Here's how the part is built. I have some questions about the finished solid (model axes, mm). A direction names the side the tool comes from. Coordinates: 2 decimals unless noted, no trailing zeros. Write each loop counter-clockwise with the first axis right and the second up, starting at its lowest first coordinate (ties: lowest second). Pieces come first, ordered by that corner, then holes.
from build123d import *

# Parameters (mm, degrees)
SKETCH_1_W                   = 100
SKETCH_1_H                   = 925
EXTRUDE_1_DEPTH              = 20
HOLE_WIZARD_M6_2_D           = 5
SKETCH_11_R                  = 42.5
CUT_EXTRUDE_1_DEPTH          = 466.624580537
HOLE_WIZARD_M8_2_D           = 9
HOLE_WIZARD_M8_2_CBORE_D     = 15
HOLE_WIZARD_M8_2_CBORE_DEPTH = 8.6
FILLET_2_R                   = 10
SKETCH_14_R                  = 42.5
CUT_EXTRUDE_2_DEPTH          = 466.624580537
HOLE_WIZARD_M6_3_D           = 5


with BuildPart() as part:
    # 草图1 → 凸台-拉伸1 (new body)
    with BuildSketch(Plane.XY):
        Rectangle(SKETCH_1_W, SKETCH_1_H)
    extrude(amount=EXTRUDE_1_DEPTH)

    # M6 螺纹孔2 (through all)
    with Locations(Plane.XY.offset(20)):
        with Locations((-18.368804754, -260.653782439), (18.368804754, -260.653782439), (18.368804754, -349.346217561), (-18.368804754, -349.346217561), (18.368804754, 349.346217561), (-18.368804754, 349.346217561), (18.368804754, 260.653782439), (-18.368804754, 260.653782439)):
            Hole(HOLE_WIZARD_M6_2_D / 2)

    # 草图11 → 切除-拉伸1 (cut, through all)
    with BuildSketch(Plane.XY.offset(20)):
        with Locations((0, -305)):
            Circle(SKETCH_11_R)
    cut_extrude_1 = extrude(amount=-CUT_EXTRUDE_1_DEPTH, mode=Mode.SUBTRACT)

    # M8 六角凹头螺钉的柱形沉头孔2 (through all)
    with Locations(Plane(origin=(0, 0, 0), x_dir=(-1, 0, 0), z_dir=(0, 0, -1))):
        with Locations((-30, -452.5), (30, -452.5), (-30, -150), (30, -150), (30, 150), (-30, 150), (30, 452.5), (-30, 452.5)):
            CounterBoreHole(HOLE_WIZARD_M8_2_D / 2, HOLE_WIZARD_M8_2_CBORE_D / 2, HOLE_WIZARD_M8_2_CBORE_DEPTH)

    # 镜向10: 切除-拉伸1 across plane
    add(cut_extrude_1.mirror(Plane.ZX), mode=Mode.SUBTRACT)

    # 圆角2
    fillet_2_edges = [part.edges().sort_by_distance(p)[0] for p in [
        (50, -462.5, 10),
        (-50, -462.5, 10),
        (-50, 462.5, 10),
        (50, 462.5, 10),
    ]]
    fillet(fillet_2_edges, radius=FILLET_2_R)

    # 草图14 → 切除-拉伸2 (cut, through all)
    with BuildSketch(Plane.XY.offset(20)):
        Circle(SKETCH_14_R)
    extrude(amount=-CUT_EXTRUDE_2_DEPTH, mode=Mode.SUBTRACT)

    # M6 螺纹孔3 (through all)
    with Locations(Plane.XY.offset(20)):
        with Locations((-18.368804754, 44.346217561), (18.368804754, 44.346217561), (18.368804754, -44.346217561), (-18.368804754, -44.346217561)):
            Hole(HOLE_WIZARD_M6_3_D / 2)


solid = part.part
1. For pin 1 Ø10.5 at (x, y) = (30, 452.5) entering from +Z; pin 2 Ø4.5 at (x, y) = (18.37, -260.65) entering from -Z; pin 3 Ø12 at (x, y) = (30, -452.5) entering from -Z, each with a flat end and sliding along its axis, tell me the tip position at first contact or that it passes through.
2. If I drill on line 1 (Y direction, x = -0.5, z = 11.5); line 2 (X direction, y = -8, z = 13.25); line 3 (Y direction, x = 22, z = 5.5), over which ranges is the centre line in solid material (lowest first)?
3. I want a section at B-B (y = 0). List the corners of the cut face in (x, z) for me.
4. On a 3-axis mill with a long thin cutter (end or side, diameter ignored), from which of +Z, -Z, +X, -X, +Y, -Y can I reach the whole of each face in a straight line? I mean faces 4 (the face through (-28.37, 445.18, 4.24)), 5 (the face through (-33.727, -25.861, 10.14)). Say none if no direction works.
5. I want a section at A-A (x = 0). List the corners of the cut face in (y, z) for me.
6. Thinking about a two-plate mould opening in Y: for faces 1 (the face through (-1, -462.5, 10)), 2 (the face through (-45, 6, 20)), 3 (the face through (-5.53, -262.86, 10.14)), which applies, pulls with the +Y half, pulls with the -Y half, needs draft (parallel to the pull), parting line crosses it, or undercut?
Response values:
1. pin 1: stops at z = 20
1. pin 2: passes through
1. pin 3: stops at z = 8.6
2. line 1: y = -462.5 to -347.5, -262.5 to -42.5, 42.5 to 262.5, 347.5 to 462.5
2. line 2: x = -50 to -41.74, 41.74 to 50
2. line 3: y = -462.5 to -341.36, -268.64 to -36.36, 36.36 to 268.64, 341.36 to 462.5
3. outline: (-50, 0) - (-42.5, 0) - (-42.5, 20) - (-50, 20) - close; (42.5, 0) - (50, 0) - (50, 20) - (42.5, 20) - close
4. face 4: -Z
4. face 5: +Z, -Z
5. outline: (-462.5, 0) - (-347.5, 0) - (-347.5, 20) - (-462.5, 20) - close; (-262.5, 0) - (-42.5, 0) - (-42.5, 20) - (-262.5, 20) - close; (42.5, 0) - (262.5, 0) - (262.5, 20) - (42.5, 20) - close; (347.5, 0) - (462.5, 0) - (462.5, 20) - (347.5, 20) - close
6. face 1: pulls with the -Y half
6. face 2: needs draft
6. face 3: undercut
